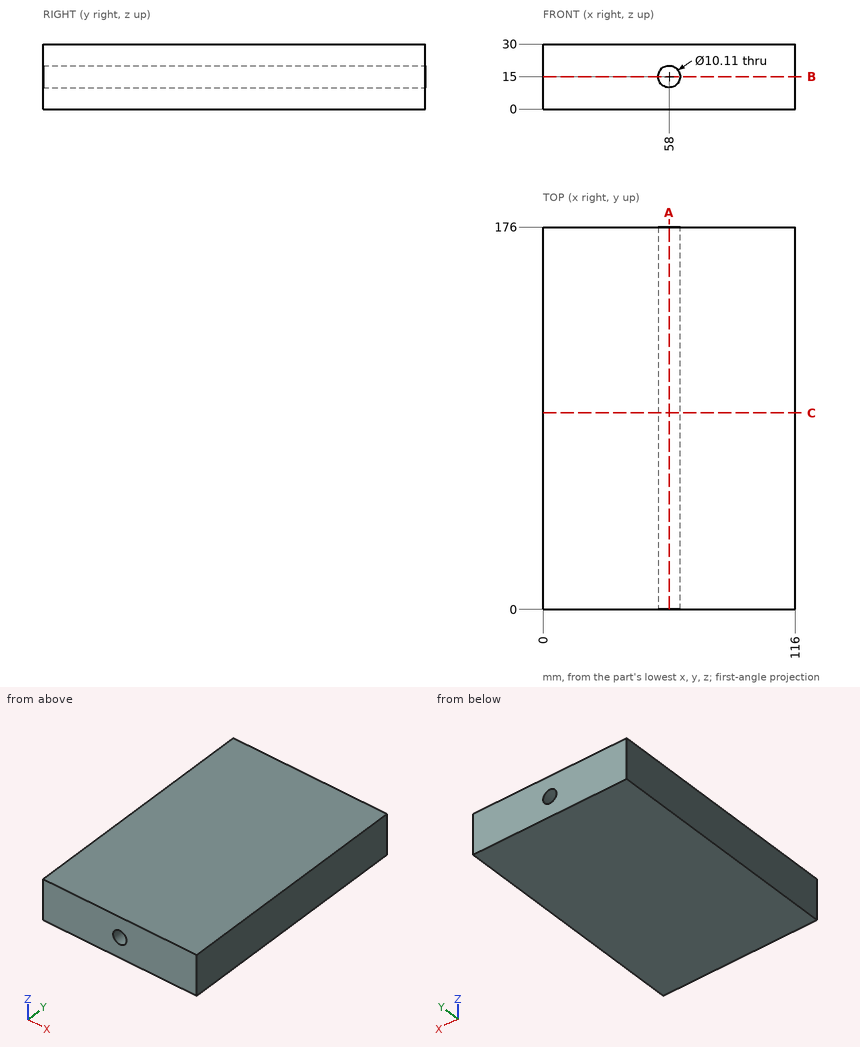
Source: three-view drawing plus pictorial views. Frame: mm from the lowest corner of the part. Coordinates: 2 decimals unless noted, no trailing zeros. Loops run counter-clockwise (first coordinate to the right, second up) from the corner with the lowest first, then second, coordinate; pieces in that order, holes last. Notation, with made-up numbers: (7, 66.5) -> (47, 66.5) arc R32 ccw to (47, 105.5) -> close; hole circle Ø10 at (27, 85.25). An arc over 180 degrees is marked (long way). One line per item, written item: value.
(1) Cut plane B-B (z = 15). Output: boundary loops of the cut face in (x, y) (3 decimals).
Answer below:
outline: (0, 0) -> (52.945, 0) -> (52.945, 176) -> (0, 176) -> close; (63.055, 0) -> (116, 0) -> (116, 176) -> (63.055, 176) -> close
(2) Cut plane C-C (y = 90.5). Output: boundary loops of the cut face in (x, z) (3 decimals), then the cut area to 3 significant figures.
Answer below:
outline: (0, 0) -> (116, 0) -> (116, 30) -> (0, 30) -> close; hole circle Ø10.11 at (58, 15)
area: 3,400 mm2
(3) Ray query, line 1 along Z through (x, y) = (58, 103) (3 decimals); line 2 along X through (y, z) = (78.5, 12.75); line 3 along X through (y, z) = (15.5, 17.5). Return the intervals inside material, ascending.
Answer below:
line 1: z = 0 to 9.945, 20.055 to 30
line 2: x = 0 to 53.47, 62.53 to 116
line 3: x = 0 to 53.61, 62.39 to 116
(4) Pin query (flat end, axial travel): pin 1 Ø1 at (x, y) = (80.5, 68) entering from -Z. Return the tip coordinate at first contact, or that it passes through.
Answer below:
pin 1: stops at z = 0
(5) Cut plane A-A (x = 58). Output: boundary loops of the cut face in (y, z) (3 decimals), then the cut area to 3 significant figures.
Answer below:
outline: (0, 0) -> (176, 0) -> (176, 9.945) -> (0, 9.945) -> close; (0, 20.055) -> (176, 20.055) -> (176, 30) -> (0, 30) -> close
area: 3,500 mm2
